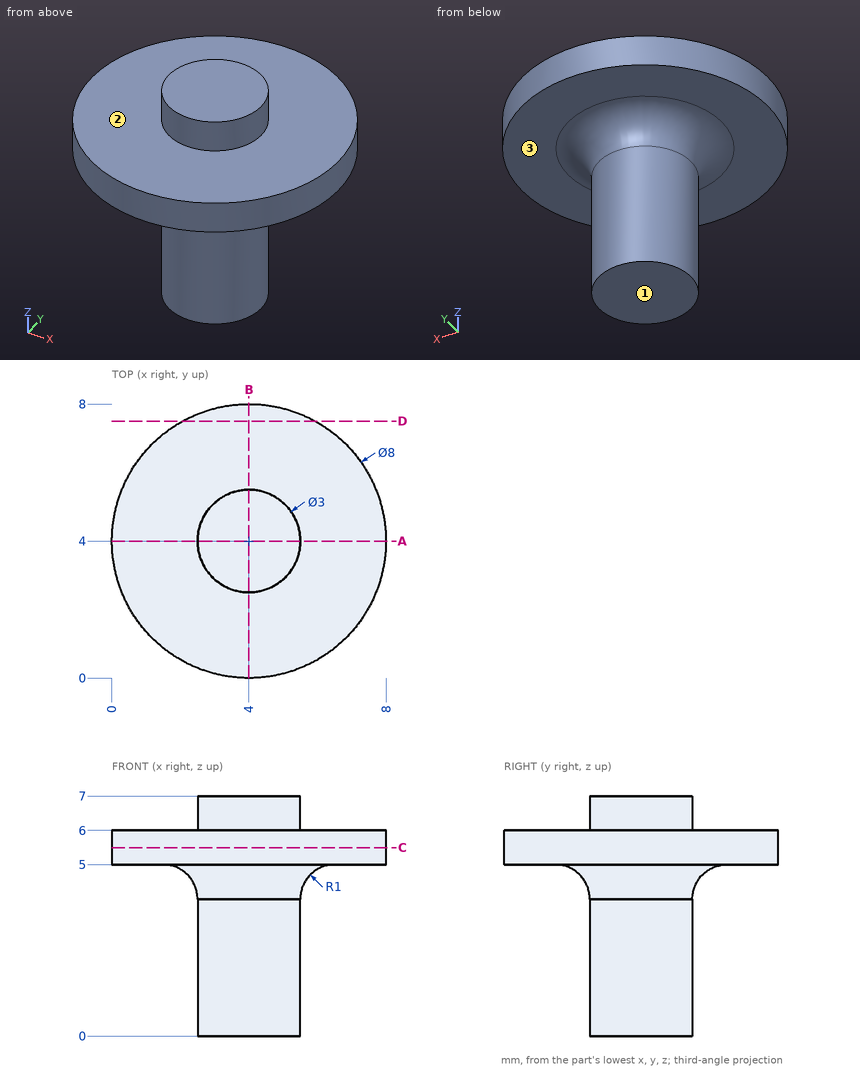
For this review, use the dimensioned drawing (mm, ordinates from the lowest corner) and the shaded views. A direction names the side the tool comes from. Round coordinates to 2 decimals unless told otherwise and drop trailing zeros. Order: outer loops, then holes, each group sorted by start corner. A loop starts at its lowest first (then second) coordinate and runs counter-clockwise, first axis right, second up. Notation, with made-up numbers: (15, 71) - (38, 71) arc R34 cw to (38, 101) - close; hole circle Ø8 at (58.25, 4.5). An arc over 180 degrees is marked (long way). Use one line per item in the form item = value.
Q1. Tool access review of the marked faces 1, 2 and 3: name each direction out of +Z, -Z, +X, -X, +Y, -Y from which nothing blocks a thin tool from reaching the whole face with its end or side.
Response values:
face_1 = -Z, +X, -X, +Y, -Y
face_2 = +Z
face_3 = -Z
Q2. Add section D-D on y = 7.5. Give the boundary of the cut face in (x, z).
Response values:
outline = (2.06, 5) - (5.94, 5) - (5.94, 6) - (2.06, 6) - close
Q3. To check wall thickness, follow line 1 (X direction, y = 4, z = 3.25); line 2 (Z direction, x = 3.5, y = 7); line 3 (X direction, y = 4.5, z = 3). State the ranges of each line that lie inside material, in increasing order.
Response values:
line_1 = 2.5 to 5.5
line_2 = 5 to 6
line_3 = 2.59 to 5.41
Q4. Add section C-C on z = 5.5. Give the boundary of the cut face in (x, y).
Response values:
outline = circle Ø8 at (4, 4)
Q5. Clearance check with flat-ended pins moving along their axes: P1, Ø3, axis at y = 2.5, z = 1, coming from the -X side; P2, Ø1, axis at x = 5.5, z = 6, coming from the -Y side; P3, Ø4, axis at x = 2, z = 1, coming from the +Y side. State where each tip first meets the part, or that it passes through.
Response values:
P1 = 2.5
P2 = 0.13
P3 = 5.5
Q6. Add section A-A on y = 4. Give the boundary of the cut face in (x, z).
Response values:
outline = (0, 5) - (1.5, 5) arc R1 cw to (2.5, 4) - (2.5, 0) - (5.5, 0) - (5.5, 4) arc R1 cw to (6.5, 5) - (8, 5) - (8, 6) - (5.5, 6) - (5.5, 7) - (2.5, 7) - (2.5, 6) - (0, 6) - close
